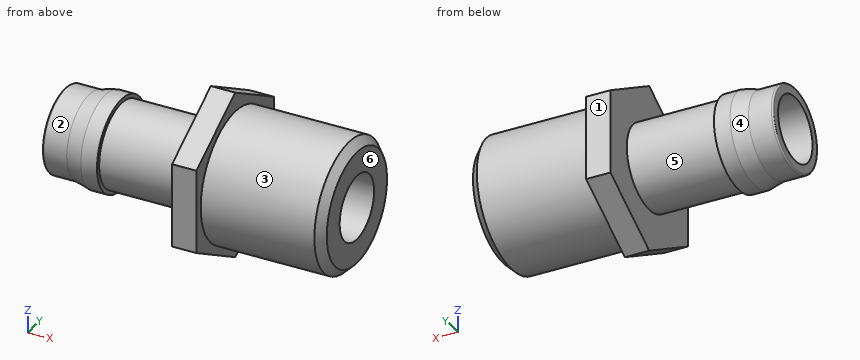
from build123d import *

# Parameters (mm, degrees)
SKETCH2_OUTSIDE_W  = 18.948
SKETCH2_OUTSIDE_H  = 18.948
CUT_EXTRUDE3_DEPTH = 10
FILLET1_R          = 0.1
CHAMFER1_SIZE      = 0.5


with BuildPart() as part:
    # Sketch1 → Revolve1 (revolve)
    with BuildSketch(Plane.XY, mode=Mode.PRIVATE) as revolve1_sk:
        Polygon((0, 2), (18, 2), (18, 4), (10.5, 4), (10.5, 6), (9, 6), (9, 2.6), (3.5, 2.6), (3.5, 2.85), (2.5, 2.85), (1.5, 2.6), (0, 2.6), align=None)
    revolve(revolve1_sk.sketch.rotate(Axis((0, 0, 0), (1, 0, 0)), 90), axis=Axis((0, 0, 0), (1, 0, 0)))

    # Sketch2 outside → Cut-Extrude3 (cut)
    with BuildSketch(Plane(origin=(10.5, 0, 0), x_dir=(0, 0, -1), z_dir=(1, 0, 0))):
        Rectangle(SKETCH2_OUTSIDE_W, SKETCH2_OUTSIDE_H)
        Polygon((2.598076211, -4.5), (5.196152423, 0), (2.598076211, 4.5), (-2.598076211, 4.5), (-5.196152423, 0), (-2.598076211, -4.5), align=None, mode=Mode.SUBTRACT)
    extrude(amount=-CUT_EXTRUDE3_DEPTH, mode=Mode.SUBTRACT)

    # Fillet1
    fillet1_edges = [part.edges().sort_by_distance(p)[0] for p in [
        (0, 0, -2.6),
    ]]
    fillet(fillet1_edges, radius=FILLET1_R)

    # Chamfer1
    chamfer1_edges = [part.edges().sort_by_distance(p)[0] for p in [
        (18, 0, -4),
    ]]
    chamfer(chamfer1_edges, length=CHAMFER1_SIZE)


solid = part.part
Model file for the job. Use its own axes, mm. Face numbers are marked on the shaded views. A direction names the side the tool comes from. Give positions to 0.01 mm unless a question says otherwise; leave off trailing zeros. Loops run counter-clockwise (first coordinate to the right, second up) from the corner with the lowest first, then second, coordinate; pieces in that order, holes last.
Item 1: Which spindle directions (+Z, -Z, +X, -X, +Y, -Y) get a long thin tool onto all of the face, cutting with end or side? Do the marked faces 1, 2 and 3. Say none if no direction does.
Check values:
face 1: +Z, -Z, +X, -X, +Y
face 2: -X
face 3: +X
Item 2: Slice it at B-B (x = 16.75). Write the cut outline in (y, z), plus the area to 3 significant figures.
Check values:
outline: circle Ø8 at (0, 0); hole circle Ø4 at (0, 0)
area: 37.7 mm2
Item 3: Drill centre lines: line 1 along Y through (x, z) = (9.5, 0); line 2 along Y through (x, z) = (7.5, 0); line 3 along X through (y, z) = (-3, -1.75). Where is each one in solid material? Low to high.
Check values:
line 1: y = -4.5 to -2, 2 to 4.5
line 2: y = -2.6 to -2, 2 to 2.6
line 3: x = 9 to 18
Item 4: Mould opens along X. For the marked faces 4, 5 and 6 say: +X half, -X half, draft (parallel to the pull), parting line (faces both ways), or undercut.
Check values:
face 4: -X half
face 5: undercut
face 6: +X half
Item 5: Drop flat-ended pins along their axis: P1, Ø2, axis at x = 8.5, y = -3, coming from the -Z side; P2, Ø1.5, axis at x = 14, z = -3.5, coming from the +Y side; P3, Ø1, axis at x = 5.5, y = 0, coming from the -Z side. Give the stop position or say it passes through.
Check values:
P1: stops at z = -3.96
P2: stops at y = 2.9
P3: stops at z = -2.6
Item 6: Slice it at A-A (z = 0). Write the cut outline in (x, y), plus the area to 3 significant figures.
Check values:
outline: (0, -2.5) arc R0.1 ccw to (0.1, -2.6) - (1.5, -2.6) - (2.5, -2.85) - (3.5, -2.85) - (3.5, -2.6) - (9, -2.6) - (9, -4.5) - (10.5, -4.5) - (10.5, -4) - (17.5, -4) - (18, -3.5) - (18, -2) - (0, -2) - close; (0, 2) - (18, 2) - (18, 3.5) - (17.5, 4) - (10.5, 4) - (10.5, 4.5) - (9, 4.5) - (9, 2.6) - (3.5, 2.6) - (3.5, 2.85) - (2.5, 2.85) - (1.5, 2.6) - (0.1, 2.6) arc R0.1 ccw to (0, 2.5) - close
area: 48.8 mm2
